Input: part model. Units: mm. Frame: model coordinates. A direction names the side the tool comes from. Coordinates: 2 decimals unless noted, no trailing zeros. Write each loop counter-clockwise with the first axis right and the second up, starting at its lowest first coordinate (ties: lowest second). Pieces come first, ordered by that corner, then holes. Notation, with made-up numbers: (-26.75, 13) - (11.25, 13) arc R31 cw to (11.25, 37) - close; hole circle Ø5 at (44, 15). An arc over 180 degrees is marked (long way). Use CSV: the item, a comma, the result in double quotes.
```python
from build123d import *

# Parameters (mm, degrees)
SKETCH1_R           = 5
BOSS_EXTRUDE1_DEPTH = 5


with BuildPart() as part:
    # Sketch1 → Boss-Extrude1 (new body)
    with BuildSketch(Plane.XY):
        with BuildLine():
            Line((9.797958971, 5), (70.202041029, 5))
            ThreePointArc((70.202041029, 5), (72.091863394, 5.370899501), (73.70131209, 6.428571429))
            ThreePointArc((73.70131209, 6.428571429), (89, 0), (73.70131209, -6.428571429))
            ThreePointArc((73.70131209, -6.428571429), (72.091863394, -5.370899501), (70.202041029, -5))
            Line((70.202041029, -5), (9.797958971, -5))
            ThreePointArc((9.797958971, -5), (7.908136606, -5.370899501), (6.29868791, -6.428571429))
            ThreePointArc((6.29868791, -6.428571429), (-9, 0), (6.29868791, 6.428571429))
            ThreePointArc((6.29868791, 6.428571429), (7.908136606, 5.370899501), (9.797958971, 5))
        make_face()
        Circle(SKETCH1_R, mode=Mode.SUBTRACT)
        with Locations((80, 0)):
            Circle(SKETCH1_R, mode=Mode.SUBTRACT)
    extrude(amount=BOSS_EXTRUDE1_DEPTH)


solid = part.part
```
(1) Ray query, probe 1 along X at (y, z) = (0.25, 1.9); probe 2 along X at (y, z) = (2.5, 3.3); probe 3 along Y at (x, z) = (0, 3.5). Return the intervals inside material, ascending. Write a range as from..to.
Check values:
probe 1,"-9..-4.99, 4.99..75.01, 84.99..89"
probe 2,"-8.65..-4.33, 4.33..75.67, 84.33..88.65"
probe 3,"-9..-5, 5..9"
(2) Cut plane D-D on y = -2. Return loops of the section in (x, z).
Check values:
outline,"(-8.77, 0) - (-4.58, 0) - (-4.58, 5) - (-8.77, 5) - close; (4.58, 0) - (75.42, 0) - (75.42, 5) - (4.58, 5) - close; (84.58, 0) - (88.77, 0) - (88.77, 5) - (84.58, 5) - close"
(3) Draft query along Y for faces 1 (the flat face through (40, 5, 2)), 2 (the cylindrical face through (84.619, -1.915, 2.465)), 3 (the cylindrical face through (7.93, -5.36, 2.46)). Return one class per face: pulls with the +Y half, pulls with the -Y half, needs draft (parallel to the pull), parting line crosses it, or undercut.
Check values:
face 1,"pulls with the +Y half"
face 2,"undercut"
face 3,"pulls with the -Y half"
(4) Cut plane A-A on x = 80. Return loops of the section in (y, z), and give its area (3 significant figures).
Check values:
outline,"(-9, 0) - (-5, 0) - (-5, 5) - (-9, 5) - close; (5, 0) - (9, 0) - (9, 5) - (5, 5) - close"
area,"40.0 mm^2"
(5) Reachability of faces 4 (the cylindrical face through (-9, 0, 2)), 5 (the cylindrical face through (7.883, 5.381, 2.465)), 6 (the flat face through (40, -5, 2)) from +Z, -Z, +X, -X, +Y, -Y: full face, straight path, thin tool, end or side. Return the list, or none.
Check values:
face 4,"+Z, -Z"
face 5,"+Z, -Z, +Y"
face 6,"+Z, -Z, -Y"
(6) Pin query (flat end, axial travel): pin 1 Ø1.5 at (x, z) = (43, 2) entering from +Y; pin 2 Ø1 at (y, z) = (-3.5, 3) entering from -X; pin 3 Ø3 at (x, z) = (21.5, 2) entering from -Y. Return the tip coordinate at first contact, or that it passes through.
Check values:
pin 1,"y = 5"
pin 2,"x = -8.49"
pin 3,"y = -5"
(7) Cut plane B-B on z = 1.1. Return loops of the section in (x, y), and give its area (3 significant figures).
Check values:
outline,"(6.3, -6.43) arc R5 cw to (9.8, -5) - (70.2, -5) arc R5 cw to (73.7, -6.43) arc R9 ccw (long way) to (73.7, 6.43) arc R5 cw to (70.2, 5) - (9.8, 5) arc R5 cw to (6.3, 6.43) arc R9 ccw (long way) to start; hole circle Ø10 at (0, 0); hole circle Ø10 at (80, 0)"
area,"984 mm^2"
(8) Cut plane C-C on y = -7.5. Return loops of the section in (x, z), and give its area (3 significant figures).
Check values:
outline,"(-4.97, 0) - (4.97, 0) - (4.97, 5) - (-4.97, 5) - close; (75.03, 0) - (84.97, 0) - (84.97, 5) - (75.03, 5) - close"
area,"99.5 mm^2"
